```python
from build123d import *

# Parameters (mm, degrees)
HOLE_WIZARD_M3_1_REACH  = 24.044
HOLE_WIZARD_M3_1_BORE_R = 1.25


with BuildPart() as part:
    # 草图1 → 旋转1 (revolve)
    with BuildSketch(Plane.XY, mode=Mode.PRIVATE) as revolve_1_sk:
        Polygon((2.5, 4), (2.5, -4), (9.5, -4), (9.5, 0.5), (7.5, 0.5), (7.5, 3), (9.5, 3), (9.5, 4), align=None)
    revolve(revolve_1_sk.sketch.rotate(Axis((0, 34.071946617, 0), (0, -1, 0)), 90), axis=Axis((0, 34.071946617, 0), (0, -1, 0)))

    # M3 螺纹孔1 bore (on position points) → M3 螺纹孔1 (cut, up to next)
    with BuildSketch(Plane(origin=(9.499977586, -1.857282502, -0.020636472), x_dir=(0.002172260237, 0, 0.99999764064), z_dir=(0.99999764064, 0, -0.002172260237)), mode=Mode.PRIVATE) as hole_wizard_m3_1_sk1:
        Circle(HOLE_WIZARD_M3_1_BORE_R)
    hole_wizard_m3_1_tool1 = extrude(hole_wizard_m3_1_sk1.sketch, amount=-HOLE_WIZARD_M3_1_REACH, mode=Mode.PRIVATE) & part.part
    add(hole_wizard_m3_1_tool1.solids().sort_by_distance((9.499978, -1.857283, -0.020636))[0], mode=Mode.SUBTRACT)


solid = part.part
```
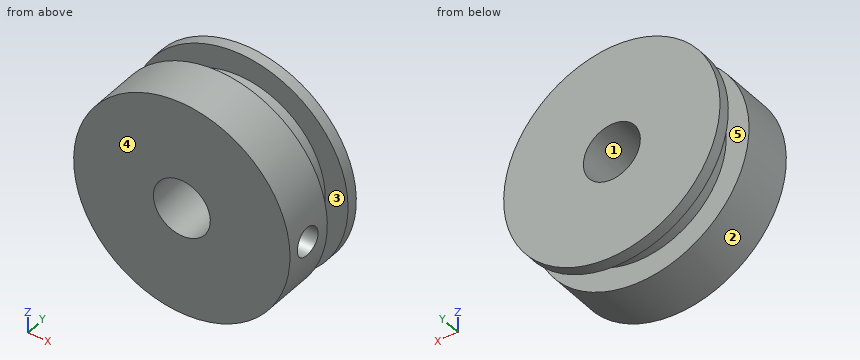
Read the model definition and answer for the solid it produces. Units are mm, in the model's axes. Face numbers are marked on the shaded views. A direction names the side the tool comes from. Coordinates: 2 decimals unless noted, no trailing zeros. Write each loop counter-clockwise with the first axis right and the second up, starting at its lowest first coordinate (ties: lowest second). Pieces come first, ordered by that corner, then holes. Notation, with made-up numbers: (42.5, -11.5) - (51.5, -11.5) arc R24 ccw to (51.5, 19.5) - close; hole circle Ø6 at (85.25, 82.5). An arc over 180 degrees is marked (long way). Answer as a JSON object with one key per item and string values. Group by question number.
1. Each of these flat-tipped pins is pushed along its axis until it touches: P1, Ø4, axis at y = 0.5, z = -4, coming from the -X side; P2, Ø3, axis at y = -0.5, z = 5.5, coming from the -X side. Where does it stop, or does it pass through?
2. Consider L1, parallel to X at y = 2.25, z = 0; L2, parallel to Y at x = 4.5, z = 7; L3, parallel to X at y = -0.25, z = 0. Determine where each line is inside the solid, lowest interval first. Write a range as [from, to].
3. A cutting plane is placed at D-D (x = -6.5). Determine the outline of the cut face in (y, z).
4. The mould has two halves that part along Z. Classify the marked faces 1, 2 and 3: +Z half, -Z half, draft (parallel to the pull), parting line (faces both ways), or undercut.
5. A cutting plane is placed at A-A (x = 0). Determine the outline of the cut face in (y, z).
6. A cutting plane is placed at B-B (y = 2.25). Determine the outline of the cut face in (x, z), plus the area to 3 significant figures.
7. A cutting plane is placed at C-C (z = -6.5). Determine the outline of the cut face in (x, y).
8. Which of the six approach directions +Z, -Z, +X, -X, +Y, -Y give full straight-line access (tool end or side, diameter ignored) to the marked faces 4 and 5?
Worked out:
{
 "1": {"P1": "stops at x = -9.29", "P2": "stops at x = -8.62"},
 "2": {"L1": "x = [-7.5, -2.5], [2.5, 7.5]", "L2": "y = [-4, 0.5], [3, 4]", "L3": "x = [-9.5, -2.5], [2.5, 9.5]"},
 "3": {"outline": "(-4, -6.93) - (0.5, -6.93) - (0.5, -3.74) - (3, -3.74) - (3, -6.93) - (4, -6.93) - (4, 6.93) - (3, 6.93) - (3, 3.74) - (0.5, 3.74) - (0.5, 6.93) - (-4, 6.93) - close"},
 "4": {"face 1": "undercut", "face 2": "parting line", "face 3": "draft"},
 "5": {"outline": "(-4, -9.5) - (0.5, -9.5) - (0.5, -7.5) - (3, -7.5) - (3, -9.5) - (4, -9.5) - (4, -2.5) - (-4, -2.5) - close; (-4, 2.5) - (4, 2.5) - (4, 9.5) - (3, 9.5) - (3, 7.5) - (0.5, 7.5) - (0.5, 9.5) - (-4, 9.5) - close"},
 "6": {"outline": "circle Ø15 at (0, 0); hole circle Ø5 at (0, 0)", "area": "157 mm²"},
 "7": {"outline": "(-6.93, -4) - (6.93, -4) - (6.93, 0.5) - (3.74, 0.5) - (3.74, 3) - (6.93, 3) - (6.93, 4) - (-6.93, 4) - (-6.93, 3) - (-3.74, 3) - (-3.74, 0.5) - (-6.93, 0.5) - close"},
 "8": {"face 4": "+Z, -Z, +X, -X, -Y", "face 5": "none"}
}
